Verification items for this drawing (mm, ordinates from the low corner). A direction names the side the tool comes from. Round coordinates to 2 decimals unless told otherwise and drop trailing zeros. Order: outer loops, then holes, each group sorted by start corner. A loop starts at its lowest first (then second) coordinate and runs counter-clockwise, first axis right, second up. Notation, with made-up numbers: (-10, -32) -> (12, -32) arc R6 ccw to (12, -26) -> close; hole circle Ø2 at (30.5, 53). An arc over 180 degrees is marked (long way). Return JSON: item names as keys, results as strings. Group by question number.
Item 1: Sectioned sample at C-C on x = 15. Record the cut outline in (y, z), plus the area to 3 significant figures.
Item 2: Sectioned sample at D-D on x = 8.5. Record the cut outline in (y, z).
Item 3: Sectioned sample at B-B on z = 5.5. Record the cut outline in (x, y).
Item 4: Access from +Z, -Z, +X, -X, +Y, -Y to the whole of each face (thin tool, end or side, straight path). Record for the marked faces 1, 2 and 3.
Item 5: Depth check by flat-ended pin: pin 1 Ø2 at (y, z) = (3.5, 6.5) entering from +X; pin 2 Ø1.5 at (x, z) = (4.5, 6.5) entering from -Y. Enter the tip coordinate at first touch or a pass-through.
Item 6: Draft check along X on the marked faces 4, 5 and 6. Enter one of: pulls with the +X half, pulls with the -X half, needs draft (parallel to the pull), parting line crosses it, or undercut.
Item 7: Scan lines: probe 1 along X at (y, z) = (15, 8.5); probe 2 along Z at (x, y) = (1.9, 15); probe 3 along Z at (x, y) = (15, 27.9). Record each from-to range of solid material in increasing order. Write a range as from..to.
Item 8: Sectioned sample at A-A on y = 15. Record the cut outline in (x, z), plus the area to 3 significant figures.
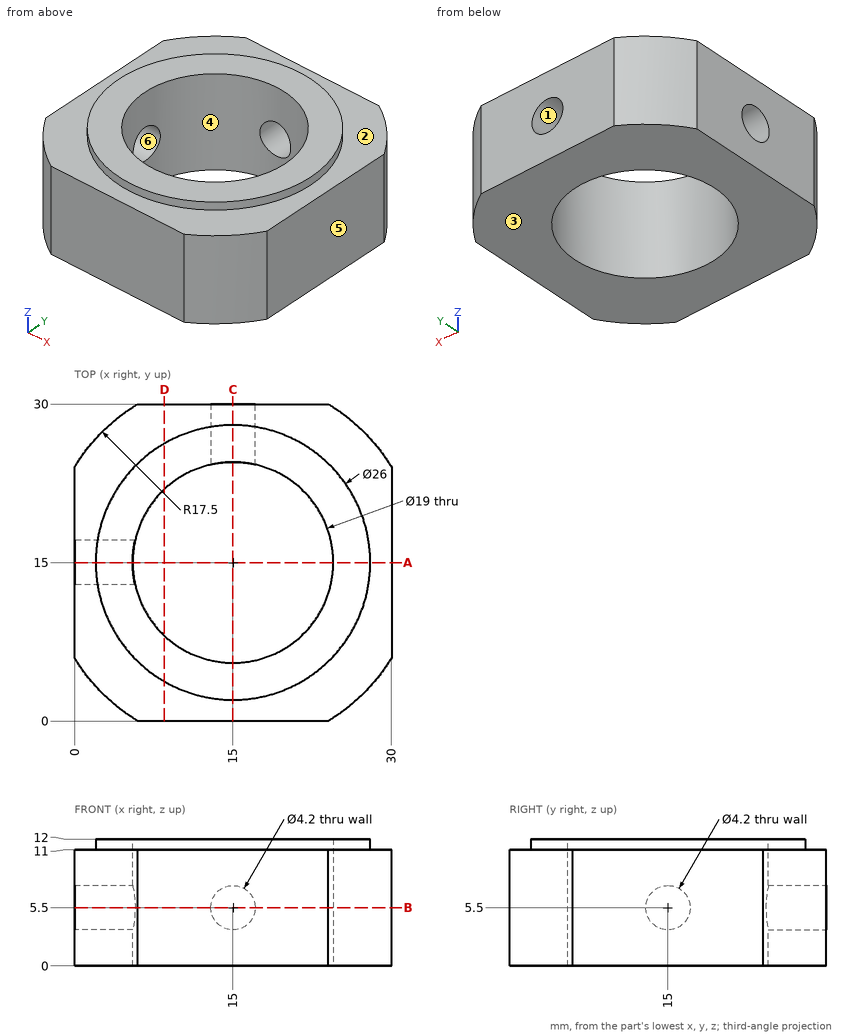
Recorded:
{
 "1": {"outline": "(0, 0) -> (5.5, 0) -> (5.5, 12) -> (2, 12) -> (2, 11) -> (0, 11) -> close; (24.5, 0) -> (30, 0) -> (30, 3.4) -> (24.5, 3.4) -> close; (24.5, 7.6) -> (30, 7.6) -> (30, 11) -> (28, 11) -> (28, 12) -> (24.5, 12) -> close", "area": "105 mm²"},
 "2": {"outline": "(0, 0) -> (8.07, 0) -> (8.07, 12) -> (3.74, 12) -> (3.74, 11) -> (0, 11) -> close; (21.93, 0) -> (30, 0) -> (30, 11) -> (26.26, 11) -> (26.26, 12) -> (21.93, 12) -> close"},
 "3": {"outline": "(0, 5.99) arc R17.5 ccw to (5.99, 0) -> (24.01, 0) arc R17.5 ccw to (30, 5.99) -> (30, 24.01) arc R17.5 ccw to (24.01, 30) -> (17.1, 30) -> (17.1, 24.26) arc R9.5 cw (long way) to (5.74, 12.9) -> (0, 12.9) -> close; (0, 17.1) -> (5.74, 17.1) arc R9.5 cw to (12.9, 24.26) -> (12.9, 30) -> (5.99, 30) arc R17.5 ccw to (0, 24.01) -> close"},
 "4": {"face 1": "+Y", "face 2": "+Z", "face 3": "-Z, +X, -X, +Y, -Y"},
 "5": {"pin 1": "x = 29", "pin 2": "y = 0.47"},
 "6": {"face 4": "undercut", "face 5": "pulls with the +X half", "face 6": "needs draft"},
 "7": {"probe 1": "0..5.5, 24.5..30", "probe 2": "0..3.4, 7.6..11", "probe 3": "0..3.4, 7.6..12"},
 "8": {"outline": "(0, 0) -> (5.5, 0) -> (5.5, 3.4) -> (0, 3.4) -> close; (0, 7.6) -> (5.5, 7.6) -> (5.5, 12) -> (2, 12) -> (2, 11) -> (0, 11) -> close; (24.5, 0) -> (30, 0) -> (30, 11) -> (28, 11) -> (28, 12) -> (24.5, 12) -> close", "area": "105 mm²"}
}
